from build123d import *

# Parameters (mm, degrees)
CUT_EXTRUDE_2_DEPTH = 6
CUT_EXTRUDE_3_DEPTH = 7.3


with BuildPart() as part:
    # 草图1 → 旋转1 (revolve)
    with BuildSketch(Plane(origin=(0, 0, 0), x_dir=(1, 0, 0), z_dir=(0, 1, 0))):
        Polygon((-25, 34), (-25, 4), (-27.5, 4), (-27.5, -156.5), (-25, -156.5), (-25, -191.5), (-12.5, -191.5), (-12.5, -217.5), (0, -217.5), (0, 34), align=None)
    revolve(axis=Axis((0, 0, 0), (0, 0, 1)))

    # 草图3 → 切除-拉伸2 (cut)
    with BuildSketch(Plane(origin=(0, -27.5, 0), x_dir=(-1, 0, 0), z_dir=(0, -1, 0))):
        with BuildLine():
            Line((8, -66.5), (8, -112.5))
            ThreePointArc((8, -112.5), (0, -120.5), (-8, -112.5))
            Line((-8, -112.5), (-8, -66.5))
            ThreePointArc((-8, -66.5), (0, -58.5), (8, -66.5))
        make_face()
    extrude(amount=-CUT_EXTRUDE_2_DEPTH, mode=Mode.SUBTRACT)

    # 草图4 → 切除-拉伸3 (cut)
    with BuildSketch(Plane(origin=(6.627052614, 14.343018289, 0), x_dir=(0.9077859676868876, -0.41943370974539124, 0), z_dir=(-0.4194337097453913, -0.9077859676868877, 0))):
        with BuildLine():
            Line((4, 219.353468604), (4, 200.5))
            ThreePointArc((4, 200.5), (0, 196.5), (-4, 200.5))
            Line((-4, 200.5), (-4, 219.353468604))
            ThreePointArc((-4, 219.353468604), (0, 223.353468604), (4, 219.353468604))
        make_face()
    extrude(amount=CUT_EXTRUDE_3_DEPTH, mode=Mode.SUBTRACT)


solid = part.part
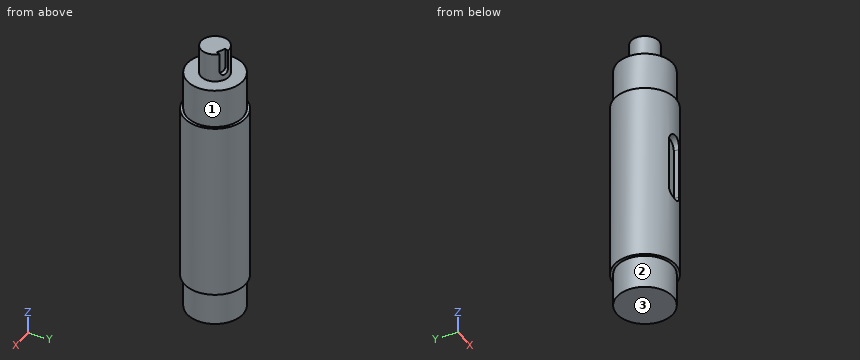
Model file for the job. Use its own axes, mm. Face numbers are marked on the shaded views. A direction names the side the tool comes from. Round coordinates to 2 decimals unless told otherwise and drop trailing zeros. Loops run counter-clockwise (first coordinate to the right, second up) from the corner with the lowest first, then second, coordinate; pieces in that order, holes last. Notation, with made-up numbers: (15.5, 62.25) - (56.5, 62.25) arc R19 ccw to (56.5, 81.25) - close; hole circle Ø10 at (35, 27.25). An arc over 180 degrees is marked (long way). Write each question's results on one line, items separated by ' | '.
(1) Saw through at C-C, the plane z = 167.5. List the corners of the cut face in (x, y).
Answer below:
outline: circle Ø50 at (0, 0)
(2) Wall check: L1, parallel to Y at x = -1, z = 33; L2, parallel to Z at x = -16, y = -3; L3, parallel to Z at x = -14.5, y = 21.5. Give the ranges that are in metal, low to high.
Answer below:
L1: y = -27.48 to 27.48 | L2: z = -34 to 191.5 | L3: z = -4 to 156.5
(3) Pin check, flat tips, straight feed: pin 1 (12 mm diameter, centred on y = -8, z = 77.5, fed in from +X); pin 2 (1.5 mm diameter, centred on x = 17.5, y = -8.5, fed in from +Z); pin 3 (5.5 mm diameter, centred on y = -24, z = 83.5, fed in from -X). Stop position of each tip, or through.
Answer below:
pin 1: stops at x = 27.43 | pin 2: stops at z = 191.5 | pin 3: stops at x = -17.46
(4) Saw through at D-D, the plane x = 22.5. List the corners of the cut face in (y, z), then the cut area to 3 significant figures.
Answer below:
outline: (-15.81, -4) - (-10.9, -4) - (-10.9, -34) - (10.9, -34) - (10.9, -4) - (15.81, -4) - (15.81, 156.5) - (10.9, 156.5) - (10.9, 191.5) - (-10.9, 191.5) - (-10.9, 156.5) - (-15.81, 156.5) - close | area: 6,490 mm^2
(5) Saw through at A-A, the plane y = 0. List the corners of the cut face in (x, z), then the cut area to 3 significant figures.
Answer below:
outline: (-27.5, -4) - (-25, -4) - (-25, -34) - (25, -34) - (25, -4) - (27.5, -4) - (27.5, 156.5) - (25, 156.5) - (25, 191.5) - (12.5, 191.5) - (12.5, 217.5) - (-12.5, 217.5) - (-12.5, 191.5) - (-25, 191.5) - (-25, 156.5) - (-27.5, 156.5) - close | area: 12,700 mm^2
(6) 3-axis set-ups, long thin cutter, end or side, ignore diameter. For the marked faces 1, 2 and 3: which of +Z, -Z, +X, -X, +Y, -Y reach the whole face in a straight line?
Answer below:
face 1: +Z | face 2: -Z | face 3: -Z, +X, -X, +Y, -Y
(7) Saw through at B-B, the plane x = -16. List the corners of the cut face in (y, z).
Answer below:
outline: (-22.37, -4) - (-19.21, -4) - (-19.21, -34) - (19.21, -34) - (19.21, -4) - (22.37, -4) - (22.37, 156.5) - (19.21, 156.5) - (19.21, 191.5) - (-19.21, 191.5) - (-19.21, 156.5) - (-22.37, 156.5) - close
